Here's the drawing with two shaded views (mm, measured from the low corner). I have some questions. Coordinates: 2 decimals unless noted, no trailing zeros. Write each loop counter-clockwise with the first axis right and the second up, starting at its lowest first coordinate (ties: lowest second). Pieces come first, ordered by that corner, then holes. Notation, with made-up numbers: M 64.25,31 L 121.25,31 A10 ccw 121.25,46 Z; hole C 48.5,4 d6. An arc over 180 degrees is marked long. Answer as CSV lines item,"result". Start each with the question number.
Item 1: If I drill on line 1 along X through (y, z) = (145, 3); line 2 along X through (y, z) = (154.5, 18.5); line 3 along Y through (x, z) = (498, 9.75), over which ranges is the centre line in solid material (lowest first)? Write a range as [from, to].
Item 2: Suppose I cut it at A-A, the plane x = 500. Write out the boundary of the cut face in (y, z), and give its area (3 significant figures).
Item 3: Suppose I cut it at B-B, the plane z = 3. Write out the boundary of the cut face in (x, y), and give its area (3 significant figures).
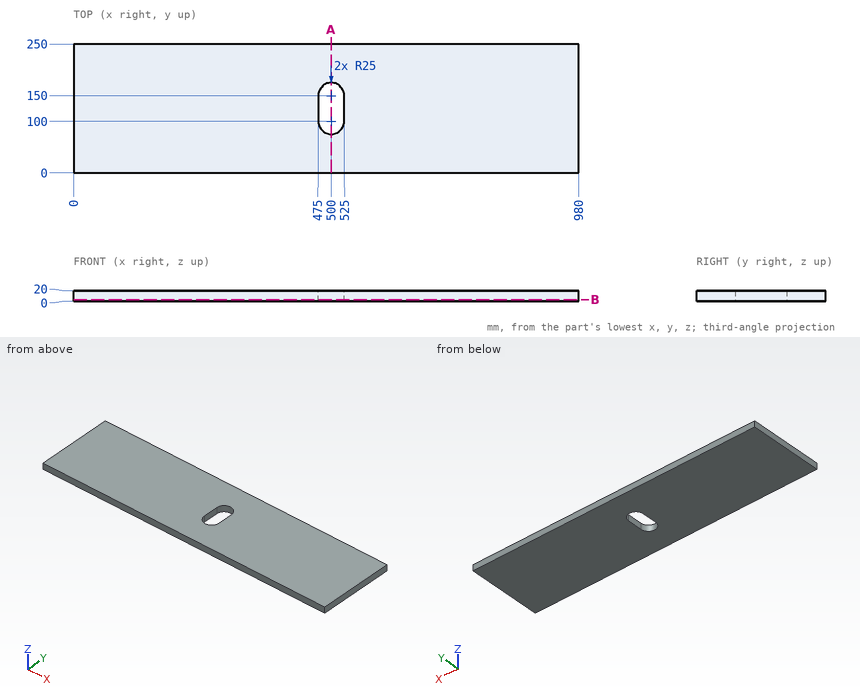
Ans:
1,line 1,"x = [0, 475], [525, 980]"
1,line 2,"x = [0, 475.41], [524.59, 980]"
1,line 3,"y = [0, 75.08], [174.92, 250]"
2,outline,"M 0,0 L 75,0 L 75,20 L 0,20 Z; M 175,0 L 250,0 L 250,20 L 175,20 Z"
2,area,"3,000 mm^2"
3,outline,"M 0,0 L 980,0 L 980,250 L 0,250 Z; hole M 475,100 A25 ccw 525,100 L 525,150 A25 ccw 475,150 Z"
3,area,"241,000 mm^2"
